from build123d import *

# Parameters (mm, degrees)
EXTRUDE_1_DEPTH        = 12
CUT_EXTRUDE_START      = -10
CUT_EXTRUDE_1_DEPTH    = 10
SKETCH_3_W             = 2
SKETCH_3_H             = 10
CUT_EXTRUDE_2_DEPTH    = 109.889852603
CUT_EXTRUDE_3_DEPTH    = 8
CUT_EXTRUDE_4_DEPTH    = 78.775317421
SKETCH_6_R             = 2.75
CUT_EXTRUDE_5_DEPTH    = 78.775317421
SKETCH_7_R             = 4.5
CUT_EXTRUDE_6_DEPTH    = 6
HOLE_WIZARD_M4_1_D     = 3.3
HOLE_WIZARD_M4_1_DEPTH = 10
HOLE_WIZARD_M4_1_TIP   = 0.991420021
HOLE_WIZARD_M4_2_D     = 3.3
HOLE_WIZARD_M4_2_DEPTH = 10
HOLE_WIZARD_M4_2_TIP   = 0.991420021
HOLE_WIZARD_M5_1_D     = 4.2


with BuildPart() as part:
    # 草图1 → 凸台-拉伸1 (new body)
    with BuildSketch(Plane.XY):
        with BuildLine():
            Line((-44, -11), (-44, -21))
            Line((-44, -21), (44, -21))
            Line((44, -21), (44, -11))
            Line((44, -11), (42, -11))
            Line((42, -11), (42, 21))
            ThreePointArc((42, 21), (0, 63), (-42, 21))
            Line((-42, 21), (-42, -11))
            Line((-42, -11), (-44, -11))
        make_face()
    extrude(amount=EXTRUDE_1_DEPTH)

    # 草图2 → 切除-拉伸1 (cut)
    with BuildSketch(Plane.XY.offset(12).offset(CUT_EXTRUDE_START)):
        with BuildLine():
            Line((-40, 21), (-40, -11))
            Line((-40, -11), (-42, -11))
            Line((-42, -11), (-42, 21))
            ThreePointArc((-42, 21), (0, 63), (42, 21))
            Line((42, 21), (42, -11))
            Line((42, -11), (40, -11))
            Line((40, -11), (40, 21))
            ThreePointArc((40, 21), (0, 61), (-40, 21))
        make_face()
    extrude(amount=CUT_EXTRUDE_1_DEPTH, mode=Mode.SUBTRACT)

    # 草图3 → 切除-拉伸2 (cut, through all)
    with BuildSketch(Plane(origin=(44, 0, 0), x_dir=(0, 0, -1), z_dir=(1, 0, 0))):
        with Locations((-11, -16)):
            Rectangle(SKETCH_3_W, SKETCH_3_H)
    extrude(amount=-CUT_EXTRUDE_2_DEPTH, mode=Mode.SUBTRACT)

    # 草图4 → 切除-拉伸3 (cut)
    with BuildSketch(Plane.XY.offset(10)):
        with BuildLine():
            Line((-40, -11), (-42, -11))
            Line((-42, -11), (-42, -16))
            ThreePointArc((-42, -16), (-41, -17), (-40, -16))
            Line((-40, -16), (-40, -11))
        make_face()
        with BuildLine():
            Line((42, -11), (42, -16))
            ThreePointArc((42, -16), (41, -17), (40, -16))
            Line((40, -16), (40, -11))
            Line((40, -11), (42, -11))
        make_face()
    extrude(amount=-CUT_EXTRUDE_3_DEPTH, mode=Mode.SUBTRACT)

    # 草图5 → 切除-拉伸4 (cut, through all)
    with BuildSketch(Plane(origin=(0, 0, 0), x_dir=(-1, 0, 0), z_dir=(0, 0, -1))):
        with BuildLine():
            Line((0, 26), (-46.263882953, 26))
            Line((-46.263882953, 26), (-46.263882953, 16))
            Line((-46.263882953, 16), (0, 16))
            ThreePointArc((0, 16), (5, 21), (0, 26))
        make_face()
    extrude(amount=-CUT_EXTRUDE_4_DEPTH, mode=Mode.SUBTRACT)

    # 草图6 → 切除-拉伸5 (cut, through all)
    with BuildSketch(Plane(origin=(0, 0, 0), x_dir=(-1, 0, 0), z_dir=(0, 0, -1))):
        with Locations((-32, -16)):
            Circle(SKETCH_6_R)
        with Locations((32, -16)):
            Circle(SKETCH_6_R)
    extrude(amount=-CUT_EXTRUDE_5_DEPTH, mode=Mode.SUBTRACT)

    # 草图7 → 切除-拉伸6 (cut)
    with BuildSketch(Plane(origin=(0, 0, 0), x_dir=(-1, 0, 0), z_dir=(0, 0, -1))):
        with Locations((-32, -16)):
            Circle(SKETCH_7_R)
        with Locations((32, -16)):
            Circle(SKETCH_7_R)
    extrude(amount=-CUT_EXTRUDE_6_DEPTH, mode=Mode.SUBTRACT)

    # M4 螺纹孔1
    with Locations(Plane(origin=(-40, 1, 7), x_dir=(0, 0, -1), z_dir=(-1, 0, 0))):
        with Locations((0, 0)):
            Hole(HOLE_WIZARD_M4_1_D / 2, depth=HOLE_WIZARD_M4_1_DEPTH)
            with Locations((0, 0, -(HOLE_WIZARD_M4_1_DEPTH + HOLE_WIZARD_M4_1_TIP / 2))):  # 118° drill point
                Cone(0, HOLE_WIZARD_M4_1_D / 2, HOLE_WIZARD_M4_1_TIP, mode=Mode.SUBTRACT)

    # M4 螺纹孔2
    with Locations(Plane(origin=(40, 1, 7.015407491), x_dir=(0, 0, 1), z_dir=(1, 0, 0))):
        with Locations((0, 0)):
            Hole(HOLE_WIZARD_M4_2_D / 2, depth=HOLE_WIZARD_M4_2_DEPTH)
            with Locations((0, 0, -(HOLE_WIZARD_M4_2_DEPTH + HOLE_WIZARD_M4_2_TIP / 2))):  # 118° drill point
                Cone(0, HOLE_WIZARD_M4_2_D / 2, HOLE_WIZARD_M4_2_TIP, mode=Mode.SUBTRACT)

    # M5 螺纹孔1 (through all)
    with Locations(Plane(origin=(0, 8.081866722, 0), x_dir=(-1, 0, 0), z_dir=(0, 0, -1))):
        with Locations((0, 0)):
            Hole(HOLE_WIZARD_M5_1_D / 2)


solid = part.part
Verification items for the finished model (mm, model axes). A direction names the side the tool comes from. Coordinates: 2 decimals unless noted, no trailing zeros. Order: outer loops, then holes, each group sorted by start corner. A loop starts at its lowest first (then second) coordinate and runs counter-clockwise, first axis right, second up. Notation, with made-up numbers: M 11.25,58.25 L 56.25,58.25 A13 ccw 56.25,80.25 Z; hole C 29.25,23.5 d11. An arc over 180 degrees is marked long. One line per item, written item: value. Start each with the question number.
Item 1: Mould release check, pull along Y, two halves, no side actions. Record for faces 6 (the flat face through (1, -16, 10)), 7 (the cylindrical face through (-1.662, 60.965, 6.93)), 8 (the cylindrical face through (-36.292, -14.648, 2.958)): pulls with the +Y half, pulls with the -Y half, needs draft (parallel to the pull), parting line crosses it, or undercut.
Item 2: Depth check by flat-ended pin: P1, Ø7, axis at x = -32, y = -16, coming from the +Z side; P2, Ø6, axis at y = 6, z = 3, coming from the -X side; P3, Ø1, axis at y = 50, z = 7, coming from the -X side; P4, Ø5, axis at x = 26.5, y = 0, coming from the -Z side. Enter the tip coordinate at first touch or a pass-through.
Item 3: Sectioned sample at C-C on y = -6. Record the cut outline in (x, z).
Item 4: Sectioned sample at A-A on x = -32. Record the cut outline in (y, z).
Item 5: Thickness scan on probe 1 along Y at (x, z) = (34, 7.25); probe 2 along Y at (x, z) = (32, 2.4); probe 3 along Y at (x, z) = (28, 5.75). Record the ranges inside material, lowest first.
Item 6: Sectioned sample at B-B on x = 32. Record the cut outline in (y, z).
Item 7: Access from +Z, -Z, +X, -X, +Y, -Y to the whole of each face (thin tool, end or side, straight path). Record for faces 1 (the flat face through (42, -13, 6)), 2 (the flat face through (1, -11, 11)), 3 (the cylindrical face through (34.93, 0.927, 8.664)), 4 (the flat face through (21, 26, 6)), 5 (the flat face through (32, -19, 6)).
Item 8: Sectioned sample at D-D on x = 21. Record the cut outline in (y, z).
Calculated:
1. face 6: needs draft
1. face 7: pulls with the +Y half
1. face 8: undercut
2. P1: z = 10
2. P2: x = -42
2. P3: x = -28.07
2. P4: z = 0
3. outline: M -42,0 L 42,0 L 42,2 L 40,2 L 40,12 L -40,12 L -40,2 L -42,2 Z
4. outline: M -21,0 L -20.5,0 L -20.5,6 L -18.75,6 L -18.75,10 L -21,10 Z; M -13.25,6 L -11.5,6 L -11.5,0 L 48.2,0 L 48.2,2 L 45,2 L 45,12 L -11,12 L -11,10 L -13.25,10 Z; hole C 1,7 d3.3
5. probe 1: -21 to -17.89, -14.11 to -0.63, 2.63 to 16, 26 to 42.07
5. probe 2: -21 to -20.5, -11.5 to 16, 26 to 45
5. probe 3: -21 to -18.06, -13.94 to 16, 26 to 49.57
6. outline: M -21,0 L -20.5,0 L -20.5,6 L -18.75,6 L -18.75,10 L -21,10 Z; M -13.25,6 L -11.5,6 L -11.5,0 L 16,0 L 16,12 L -11,12 L -11,10 L -13.25,10 Z; M 26,0 L 48.2,0 L 48.2,2 L 45,2 L 45,12 L 26,12 Z; hole C 1,7.02 d3.3
7. face 1: +Z, +Y
7. face 2: +Z, +X, -X, -Y
7. face 3: +X
7. face 4: +Z, -Z, +X
7. face 5: -Z
8. outline: M -21,0 L 16,0 L 16,12 L -11,12 L -11,10 L -21,10 Z; M 26,0 L 57.37,0 L 57.37,2 L 55.04,2 L 55.04,12 L 26,12 Z
